```python
from build123d import *

# Parameters (mm, degrees)
CUT_EXTRUDE1_DEPTH      = 100.081673268
CUT_EXTRUDE1_DEPTH_BACK = 100.081673268
SKETCH2_W               = 1
SKETCH2_H               = 10
M6_TAPPED_HOLE1_D       = 5
M6_TAPPED_HOLE1_DEPTH   = 12
M6_TAPPED_HOLE1_TIP     = 1.502151548


with BuildPart() as part:
    # Sketch1 → Revolve1 (revolve)
    with BuildSketch(Plane.XY):
        Polygon((0, 14.170965918), (0, -98.829034082), (-4, -98.829034082), (-4, -88.829034082), (-3, -88.829034082), (-3, -85.829034082), (-5, -85.829034082), (-5, 14.170965918), align=None)
    revolve(axis=Axis((0, 14.170965918, 0), (0, -1, 0)))

    # Sketch2 → Cut-Extrude1 (cut, two sides: drawn at the far end of the back side and taken through both)
    with BuildSketch(Plane.XY.offset(-CUT_EXTRUDE1_DEPTH_BACK)):
        with Locations((-4.5, -60.829034082)):
            Rectangle(SKETCH2_W, SKETCH2_H)
        with Locations((4.5, -60.829034082)):
            Rectangle(SKETCH2_W, SKETCH2_H)
    extrude(amount=CUT_EXTRUDE1_DEPTH + CUT_EXTRUDE1_DEPTH_BACK, mode=Mode.SUBTRACT)

    # M6 Tapped Hole1
    with Locations(Plane(origin=(0, 14.170965918, 0), x_dir=(1, 0, 0), z_dir=(0, 1, 0))):
        with Locations((0, 0)):
            Hole(M6_TAPPED_HOLE1_D / 2, depth=M6_TAPPED_HOLE1_DEPTH)
            with Locations((0, 0, -(M6_TAPPED_HOLE1_DEPTH + M6_TAPPED_HOLE1_TIP / 2))):  # 118° drill point
                Cone(0, M6_TAPPED_HOLE1_D / 2, M6_TAPPED_HOLE1_TIP, mode=Mode.SUBTRACT)


solid = part.part
```
The model under review builds one solid part; all positions refer to its coordinate system, in mm. A direction names the side the tool comes from. Give positions to 0.01 mm unless a question says otherwise; leave off trailing zeros. Write each loop counter-clockwise with the first axis right and the second up, starting at its lowest first coordinate (ties: lowest second). Pieces come first, ordered by that corner, then holes. Notation, with made-up numbers: M 41.5,24 L 97.5,24 A8 cw 97.5,36 Z; hole C 24.5,35.25 d8. An arc over 180 degrees is marked long. Write each question's results on one line, items separated by ' | '. Start each with the question number.
1. For probe 1 along Z at (x, y) = (0, 8.75); probe 2 along Y at (x, z) = (2.75, -1.5); probe 3 along X at (y, z) = (-21.5, -4), list the stretches that pass through material, from the lowest coordinate up. Write a range as [from, to].
2. Insertion check: pin 1 Ø4 at (x, y) = (-3.5, -47.5) entering from +Z; pin 2 Ø5 at (y, z) = (-59.5, -0.5) entering from +X; pin 3 Ø0.8 at (x, z) = (4.5, -1.5) entering from -Y. Each pin has a flat end and moves straight along its axis. Give the tip position at first contact, or say it passes through.
3. Mouldability with a two-part tool opening along Z and no side actions: class faces 1 (the cylindrical face through (0.54, 8.09, 2.44)), 2 (the flat face through (0, -98.829, 0)), 3 (the cylindrical face through (0.867, -93.759, 3.905)) as released by +Z, released by -Z, zero draft, split by the parting line, or undercut.
4. For faces 4 (the conical face through (-0.094, 0.93, 0.424)), 5 (the cylindrical face through (5, -35, 0)), 6 (the flat face through (4, -61, 0)), 7 (the flat face through (-1, -88.829, -3)), 8 (the flat face through (-4, -61, 0)), list the 3-axis set-ups (+Z, -Z, +X, -X, +Y, -Y) from which the entire face can be reached by the end or side of a thin tool; tool diameter is ignored.
5. We need section A-A (y = -52). Write out the cut boundary in (x, z), and give its area (3 significant figures).
Results found:
1) probe 1: z = [-5, -2.5], [2.5, 5] | probe 2: y = [-98.83, -88.83], [-85.83, 14.17] | probe 3: x = [-3, 3]
2) pin 1: stops at z = 4.77 | pin 2: stops at x = 4 | pin 3: stops at y = -85.83
3) face 1: undercut | face 2: zero draft | face 3: split by the parting line
4) face 4: +Y | face 5: +Y, -Y | face 6: +Z, -Z, +X | face 7: none | face 8: +Z, -Z, -X
5) outline: C 0,0 d10 | area: 78.5 mm^2
